For this review, use the dimensioned drawing (mm, ordinates from the lowest corner) and the shaded views. Coordinates: 2 decimals unless noted, no trailing zeros. Write each loop counter-clockwise with the first axis right and the second up, starting at its lowest first coordinate (ties: lowest second). Pieces come first, ordered by that corner, then holes. Notation, with made-up numbers: (4, 32) - (20, 32) arc R21 ccw to (20, 53) - close; hole circle Ø10 at (39, 46.5). An arc over 180 degrees is marked (long way). Put each result on its own line as item: value.
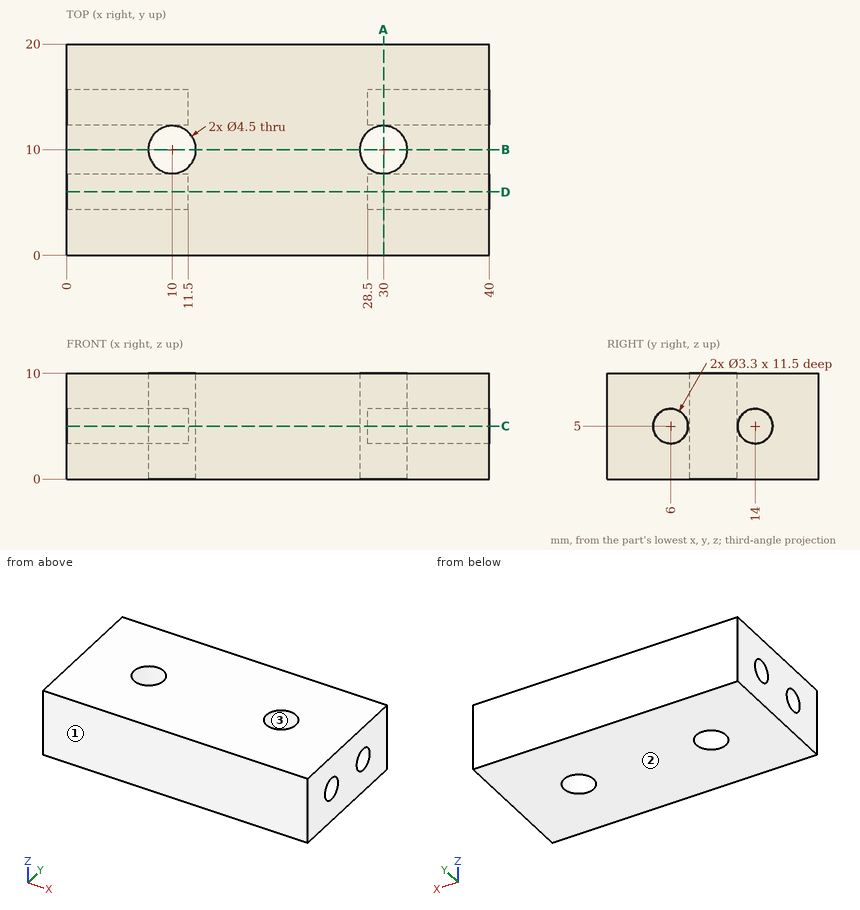
1. Consider section A-A on x = 30. State the section outline as (y, z) points.
Determined:
outline: (0, 0) - (7.75, 0) - (7.75, 10) - (0, 10) - close; (12.25, 0) - (20, 0) - (20, 10) - (12.25, 10) - close; hole circle Ø3.3 at (6, 5); hole circle Ø3.3 at (14, 5)
2. The part is to be moulded in two halves that separate along Y. For the marked faces 1, 2 and 3, say which applies: +Y half, -Y half, draft (parallel to the pull), parting line (faces both ways), or undercut.
Determined:
face 1: -Y half
face 2: draft
face 3: undercut
3. Consider section D-D on y = 6. State the section outline as (x, z) points, plus the area to 3 significant figures.
Determined:
outline: (0, 0) - (40, 0) - (40, 3.35) - (28.5, 3.35) - (28.5, 6.65) - (40, 6.65) - (40, 10) - (0, 10) - (0, 6.65) - (11.5, 6.65) - (11.5, 3.35) - (0, 3.35) - close
area: 324 mm^2
4. Consider section B-B on y = 10. State the section outline as (x, z) points.
Determined:
outline: (0, 0) - (7.75, 0) - (7.75, 10) - (0, 10) - close; (12.25, 0) - (27.75, 0) - (27.75, 10) - (12.25, 10) - close; (32.25, 0) - (40, 0) - (40, 10) - (32.25, 10) - close
5. To check wall thickness, follow probe 1 along Y at (x, z) = (32.75, 5); probe 2 along Z at (x, y) = (4, 14); probe 3 along Y at (x, z) = (10, 7). State the ranges of each line that lie inside material, in increasing order.
Determined:
probe 1: y = 0 to 4.35, 7.65 to 12.35, 15.65 to 20
probe 2: z = 0 to 3.35, 6.65 to 10
probe 3: y = 0 to 7.75, 12.25 to 20
6. For pin 1 Ø3 at (y, z) = (14, 5) entering from -X; pin 2 Ø1.6 at (y, z) = (14.5, 4.5) entering from +X; pin 3 Ø3.5 at (x, y) = (30, 10) entering from -Z, all flat-tipped, find the tip position at first contact; note any pin that passes through.
Determined:
pin 1: stops at x = 11.5
pin 2: stops at x = 28.5
pin 3: passes through
7. Consider section C-C on z = 5. State the section outline as (x, y) points.
Determined:
outline: (0, 0) - (40, 0) - (40, 4.35) - (28.5, 4.35) - (28.5, 7.65) - (40, 7.65) - (40, 12.35) - (28.5, 12.35) - (28.5, 15.65) - (40, 15.65) - (40, 20) - (0, 20) - (0, 15.65) - (11.5, 15.65) - (11.5, 12.35) - (0, 12.35) - (0, 7.65) - (11.5, 7.65) - (11.5, 4.35) - (0, 4.35) - close; hole circle Ø4.5 at (10, 10); hole circle Ø4.5 at (30, 10)
